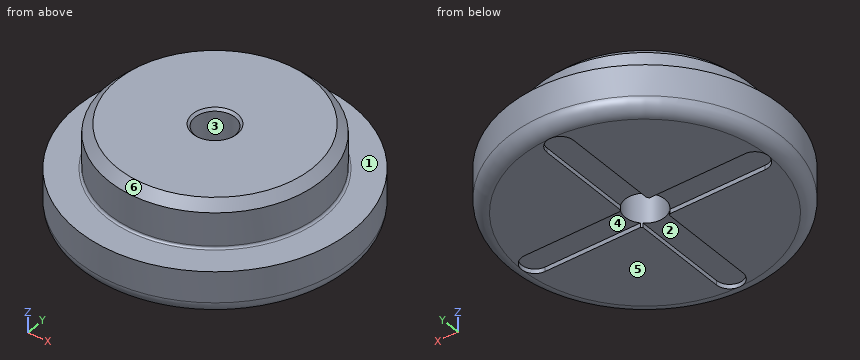
from build123d import *

# Parameters (mm, degrees)
SKETCH_1_R            = 31
EXTRUDE_1_DEPTH       = 10
SKETCH_2_R            = 24
EXTRUDE_2_DEPTH       = 10
CHAMFER_1_SIZE        = 2
FILLET_1_R            = 3
M10X1_0_1_D           = 9
M10X1_0_1_DEPTH       = 25
M10X1_0_1_CSINK_D     = 10.05
M10X1_0_1_CSINK_ANGLE = 90
M10X1_0_1_TIP         = 2.703872786
CUT_EXTRUDE_1_DEPTH   = 1
CUT_EXTRUDE_2_DEPTH   = 1
FILLET_2_R            = 0.5


with BuildPart() as part:
    # 草图1 → 凸台-拉伸1 (new body)
    with BuildSketch(Plane.XY):
        Circle(SKETCH_1_R)
    extrude(amount=EXTRUDE_1_DEPTH)

    # 草图2 → 凸台-拉伸2 (add)
    with BuildSketch(Plane.XY.offset(10)):
        Circle(SKETCH_2_R)
    extrude(amount=EXTRUDE_2_DEPTH)

    # 倒角1
    chamfer_1_edges = [part.edges().sort_by_distance(p)[0] for p in [
        (-24, 0, 20),
    ]]
    chamfer(chamfer_1_edges, length=CHAMFER_1_SIZE)

    # 圆角1
    fillet_1_edges = [part.edges().sort_by_distance(p)[0] for p in [
        (-31, 0, 0),
    ]]
    fillet(fillet_1_edges, radius=FILLET_1_R)

    # M10x1.0 螺纹孔1
    with Locations(Plane.XY.offset(20)):
        with Locations((0, 0)):
            CounterSinkHole(M10X1_0_1_D / 2, M10X1_0_1_CSINK_D / 2, depth=M10X1_0_1_DEPTH, counter_sink_angle=M10X1_0_1_CSINK_ANGLE)
            with Locations((0, 0, -(M10X1_0_1_DEPTH + M10X1_0_1_TIP / 2))):  # 118° drill point
                Cone(0, M10X1_0_1_D / 2, M10X1_0_1_TIP, mode=Mode.SUBTRACT)

    # 草图4 → 切除-拉伸1 (cut)
    with BuildSketch(Plane(origin=(0, 0, 0), x_dir=(-1, 0, 0), z_dir=(0, 0, -1))):
        with BuildLine():
            Line((-3, -25), (-3, 25))
            ThreePointArc((-3, 25), (0, 28), (3, 25))
            Line((3, 25), (3, -25))
            ThreePointArc((3, -25), (0, -28), (-3, -25))
        make_face()
    extrude(amount=-CUT_EXTRUDE_1_DEPTH, mode=Mode.SUBTRACT)

    # 草图5 → 切除-拉伸2 (cut)
    with BuildSketch(Plane(origin=(0, 0, 0), x_dir=(-1, 0, 0), z_dir=(0, 0, -1))):
        with BuildLine():
            Line((-25, 3), (25, 3))
            ThreePointArc((25, 3), (28, 0), (25, -3))
            Line((25, -3), (-25, -3))
            ThreePointArc((-25, -3), (-28, 0), (-25, 3))
        make_face()
    extrude(amount=-CUT_EXTRUDE_2_DEPTH, mode=Mode.SUBTRACT)

    # 圆角2
    fillet_2_edges = [part.edges().sort_by_distance(p)[0] for p in [
        (-24, 0, 10),
    ]]
    fillet(fillet_2_edges, radius=FILLET_2_R)


solid = part.part
Can you work these out from the model? Positions are in its coordinate system, mm. Face numbers are marked on the shaded views. A direction names the side the tool comes from. Give positions to 0.01 mm unless a question says otherwise; leave off trailing zeros. Loops run counter-clockwise (first coordinate to the right, second up) from the corner with the lowest first, then second, coordinate; pieces in that order, holes last. Notation, with made-up numbers: (52.5, 14.5) -> (57.5, 14.5) arc R28 cw to (57.5, 36.5) -> close; hole circle Ø1 at (33.25, 73.5). An arc over 180 degrees is marked (long way). Use one line per item in the form item = value.
1) If we section it at B-B (z = 15.5): Please give me the cut outline in (x, y).
Answers:
outline = circle Ø48 at (0, 0); hole circle Ø9 at (0, 0)
2) We'd pull the mould along Y, two halves only. Please class the marked faces 4, 5 and 6: released by +Y, released by -Y, zero draft, split by the parting line, or undercut.
Answers:
face_4 = undercut
face_5 = zero draft
face_6 = split by the parting line
3) If we section it at A-A (z = 7.25): Please give me the cut outline in (x, y), plus the area to 3 significant figures.
Answers:
outline = circle Ø62 at (0, 0); hole circle Ø9 at (0, 0)
area = 2,960 mm²
4) For the marked faces 1, 2 and 3, which set-ups out of +Z, -Z, +X, -X, +Y, -Y let a thin tool reach every point of the face, with its end or its side?
Answers:
face_1 = +Z
face_2 = -Z
face_3 = +Z, -Z
5) I need wall thicknesses on line 1 along Y through (x, z) = (0, 9); line 2 along Z through (x, y) = (-20, 15); line 3 along Y through (x, z) = (1.5, 4). Which ranges of each line are inside material? Lowest first, please.
Answers:
line_1 = -31 to -4.5, 4.5 to 31
line_2 = 0 to 10
line_3 = -30.96 to -4.24, 4.24 to 30.96
6) Will these pins go through, and if not, where does the flat tip stop? pin 1 (5 mm diameter, centred on x = 1.5, y = -20.5, fed in from -Z); pin 2 (4 mm diameter, centred on x = -18, z = 17, fed in from +Y); pin 3 (12 mm diameter, centred on x = 23, y = -19.5, fed in from +Z); pin 4 (1 mm diameter, centred on x = -1.5, z = 14.5, fed in from -Y).
Answers:
pin_1 = 0
pin_2 = 17.89
pin_3 = 10.14
pin_4 = -23.98
